Geometry check sheet. Reference: the model listing, model coordinates, mm. Give positions to 0.01 mm unless a question says otherwise; leave off trailing zeros. Loops run counter-clockwise (first coordinate to the right, second up) from the corner with the lowest first, then second, coordinate; pieces in that order, holes last. Notation, with made-up numbers: (0, 43.5) - (55, 43.5) arc R31 cw to (55, 77.5) - close; hole circle Ø7 at (85, 84). An arc over 180 degrees is marked (long way). Use a Markdown table: item, result. Add a question column.
1. Draft check along Y on faces 1 (the cylindrical face through (5.208, 21.586, 0.739)), 2 (the flat face through (0, -25, 1)), 3 (the cylindrical face through (-4.792, 21.586, 0.739)), 4 (the flat face through (8.5, 24.5, 0.7)). Enter one of: pulls with the +Y half, pulls with the -Y half, needs draft (parallel to the pull), parting line crosses it, or undercut.
2. Cross-section at C-C on z = 0.35. Enter the section's corners in (x, y).
3. Material ranges on L1, parallel to Y at x = 5, z = 0.65; L2, parallel to Y at x = 6, z = 0.4, recorded low to high.
4. Cross-section at A-A on y = 20. Enter the section's corners in (x, z).
5. Cross-section at B-B on x = 5. Enter the section's corners in (y, z).
from build123d import *

# Parameters (mm, degrees)
SKETCH1_W                      = 18
SKETCH1_H                      = 50
BOSS_EXTRUDE1_DEPTH            = 1.5
F_3_2_3_2_DIAMETER_HOLE1_D     = 3.2
F_3_2_3_2_DIAMETER_HOLE1_DEPTH = 12
F_3_2_3_2_DIAMETER_HOLE1_TIP   = 0.96137699
CHAMFER1_SIZE                  = 1


with BuildPart() as part:
    # Sketch1 → Boss-Extrude1 (new body)
    with BuildSketch(Plane.XY):
        Rectangle(SKETCH1_W, SKETCH1_H)
    extrude(amount=BOSS_EXTRUDE1_DEPTH)

    # Ø3.2 (3.2) Diameter Hole1
    with Locations(Plane.XY.offset(1.5)):
        with Locations((-5, 20), (5, 20)):
            Hole(F_3_2_3_2_DIAMETER_HOLE1_D / 2, depth=F_3_2_3_2_DIAMETER_HOLE1_DEPTH)
            with Locations((0, 0, -(F_3_2_3_2_DIAMETER_HOLE1_DEPTH + F_3_2_3_2_DIAMETER_HOLE1_TIP / 2))):  # 118° drill point
                Cone(0, F_3_2_3_2_DIAMETER_HOLE1_D / 2, F_3_2_3_2_DIAMETER_HOLE1_TIP, mode=Mode.SUBTRACT)

    # Chamfer1
    chamfer1_edges = [part.edges().sort_by_distance(p)[0] for p in [
        (9, -25, 0.75),
        (-9, -25, 0.75),
        (-9, 25, 0.75),
        (9, 25, 0.75),
    ]]
    chamfer(chamfer1_edges, length=CHAMFER1_SIZE)


solid = part.part
Values found:
| question | item | result |
|---|---|---|
| 1 | face 1 | undercut |
| 1 | face 2 | pulls with the -Y half |
| 1 | face 3 | undercut |
| 1 | face 4 | pulls with the +Y half |
| 2 | outline | (-9, -24) - (-8, -25) - (8, -25) - (9, -24) - (9, 24) - (8, 25) - (-8, 25) - (-9, 24) - close; hole circle Ø3.2 at (-5, 20); hole circle Ø3.2 at (5, 20) |
| 3 | L1 | y = -25 to 18.4, 21.6 to 25 |
| 3 | L2 | y = -25 to 18.75, 21.25 to 25 |
| 4 | outline | (-9, 0) - (-6.6, 0) - (-6.6, 1.5) - (-9, 1.5) - close; (-3.4, 0) - (3.4, 0) - (3.4, 1.5) - (-3.4, 1.5) - close; (6.6, 0) - (9, 0) - (9, 1.5) - (6.6, 1.5) - close |
| 5 | outline | (-25, 0) - (18.4, 0) - (18.4, 1.5) - (-25, 1.5) - close; (21.6, 0) - (25, 0) - (25, 1.5) - (21.6, 1.5) - close |
